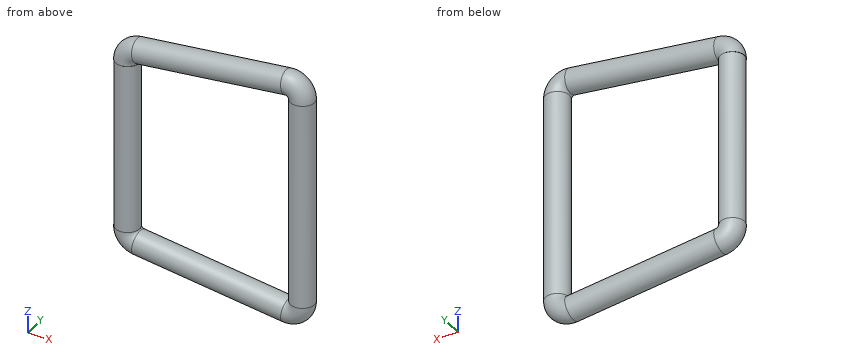
from build123d import *

# Parameters (mm, degrees)
EXTRUDE_1_DEPTH      = 8.65
EXTRUDE_1_DEPTH_BACK = 8.65
SKETCH_1_R           = 1
SKETCH_2_R           = 1
REVOLVE_1_ANGLE      = 97
SKETCH_3_R           = 1
REVOLVE_2_ANGLE      = 97
SKETCH_4_R           = 1
EXTRUDE_2_DEPTH      = 12.65745
SKETCH_5_R           = 1
EXTRUDE_3_DEPTH      = 12.65745
SKETCH_6_R           = 1
REVOLVE_3_ANGLE      = 83
SKETCH_7_R           = 1
REVOLVE_4_ANGLE      = 83
EXTRUDE_4_DEPTH      = 7.10745
EXTRUDE_4_DEPTH_BACK = 7.10745
SKETCH_8_R           = 1


with BuildPart() as part:
    # 草图1 → 凸台-拉伸1 (new, two sides: drawn at the far end of the back side and taken through both)
    with BuildSketch(Plane.XY.offset(-EXTRUDE_1_DEPTH_BACK)):
        with Locations((8.57, 0)):
            Circle(SKETCH_1_R)
    extrude(amount=EXTRUDE_1_DEPTH + EXTRUDE_1_DEPTH_BACK)

    # 草图2 → 旋转1 (revolve)
    with BuildSketch(Plane(origin=(0, 0, -8.65), x_dir=(-1, 0, 0), z_dir=(0, 0, -1))):
        with Locations(Location((-8.57, 0, 0), (0, 0, 180))):
            Circle(SKETCH_2_R)
    revolve(axis=Axis((7.47, 1, -8.65), (0, 1, 0)), revolution_arc=REVOLVE_1_ANGLE)

    # 草图3 → 旋转2 (revolve)
    with BuildSketch(Plane.XY.offset(8.65)):
        with Locations((8.57, 0)):
            Circle(SKETCH_3_R)
    revolve(axis=Axis((7.47, -1, 8.65), (0, -1, 0)), revolution_arc=REVOLVE_2_ANGLE)

    # 草图4 → 凸台-拉伸2 (add)
    with BuildSketch(Plane(origin=(8.405366736, 0, -1.032049264), x_dir=(0.12186934340514718, 0, 0.9925461516413221), z_dir=(-0.9925461516413221, 0, 0.12186934340514718))):
        with Locations(Location((-8.775160216, 0, 0), (0, 0, 180))):
            Circle(SKETCH_4_R)
    extrude(amount=EXTRUDE_2_DEPTH)

    # 草图5 → 凸台-拉伸3 (add)
    with BuildSketch(Plane(origin=(8.405366736, 0, 1.032049264), x_dir=(-0.12186934340514718, 0, 0.9925461516413221), z_dir=(-0.9925461516413221, 0, -0.12186934340514718))):
        with Locations((8.775160216, 0)):
            Circle(SKETCH_5_R)
    extrude(amount=EXTRUDE_3_DEPTH)

    # 草图6 → 旋转3 (revolve)
    with BuildSketch(Plane(origin=(-4.157736551, 0, 0.510505857), x_dir=(0.12186934340514717, 0, 0.9925461516413221), z_dir=(-0.9925461516413221, 0, 0.12186934340514717))):
        with Locations(Location((-8.775160216, 0, 0), (0, 0, 180))):
            Circle(SKETCH_6_R)
    revolve(axis=Axis((-5.093103287, 1, -7.107444879), (0, 1, 0)), revolution_arc=REVOLVE_3_ANGLE)

    # 草图7 → 旋转4 (revolve)
    with BuildSketch(Plane(origin=(-4.157736551, 0, -0.510505857), x_dir=(-0.12186934340514716, 0, 0.9925461516413221), z_dir=(-0.9925461516413221, 0, -0.12186934340514716))):
        with Locations((8.775160216, 0)):
            Circle(SKETCH_7_R)
    revolve(axis=Axis((-5.093103287, -1, 7.107444879), (0, -1, 0)), revolution_arc=REVOLVE_4_ANGLE)

    # 草图8 → 凸台-拉伸4 (add, two sides: drawn at the far end of the back side and taken through both)
    with BuildSketch(Plane.XY.offset(-EXTRUDE_4_DEPTH_BACK)):
        with Locations(Location((-6.177315, 0, 0), (0, 0, 90.452305782))):
            Circle(SKETCH_8_R)
    extrude(amount=EXTRUDE_4_DEPTH + EXTRUDE_4_DEPTH_BACK)


solid = part.part
CAD build for the part. Positions are in the model's coordinates, mm. Round coordinates to 2 decimals unless told otherwise and drop trailing zeros. Write each loop counter-clockwise with the first axis right and the second up, starting at its lowest first coordinate (ties: lowest second). Pieces come first, ordered by that corner, then holes. Notation, with made-up numbers: M -12.5,-1.5 L 46.5,-1.5 A20 ccw 46.5,28.5 Z; hole C 41,49 d4. An arc over 180 degrees is marked long. Use a Markdown table: item, result. Add a question column.
1. Drill centre lines: probe 1 along Z at (x, y) = (0, 0.4); probe 2 along X at (y, z) = (0.8, 1.75); probe 3 along X at (y, z) = (0.55, -4.75). Where is each one in solid material? Low to high.
2. Slice it at B-B on z = 5.5. Give the cut face in (x, y), then the cut area to 3 significant figures.
3. Flat gauge pins, fed straight in: P1, Ø1, axis at x = -1, y = -0.5, coming from the +Z side; P2, Ø0.8, axis at x = -6.5, y = 0, coming from the -Z side; P3, Ø0.5, axis at x = -5.5, y = -0.5, coming from the +Z side. Where does each tip first touch, or does it go through?
Reply:
| question | item | result |
|---|---|---|
| 1 | probe 1 | z = -9.76 to -7.92, 7.92 to 9.76 |
| 1 | probe 2 | x = -6.78 to -5.58, 7.97 to 9.17 |
| 1 | probe 3 | x = -7.01 to -5.34, 7.73 to 9.41 |
| 2 | outline | C -6.18,0 d2; C 8.57,0 d2 |
| 2 | area | 6.28 mm^2 |
| 3 | P1 | stops at z = 9.76 |
| 3 | P2 | stops at z = -8.95 |
| 3 | P3 | stops at z = 9.15 |
